Source: CAD feature listing. Evaluate the final solid. Frame: model axes, mm. Give positions to 0.01 mm unless a question says otherwise; leave off trailing zeros. Write each loop counter-clockwise with the first axis right and the second up, starting at its lowest first coordinate (ties: lowest second). Pieces come first, ordered by that corner, then holes. Notation, with made-up numbers: M 20,-6 L 44,-6 A8 ccw 44,-1 Z; hole C 74.5,67.25 d1. An arc over 180 degrees is marked long. Use CSV: the item, a comma, the result in double quotes. Start each with the question number.
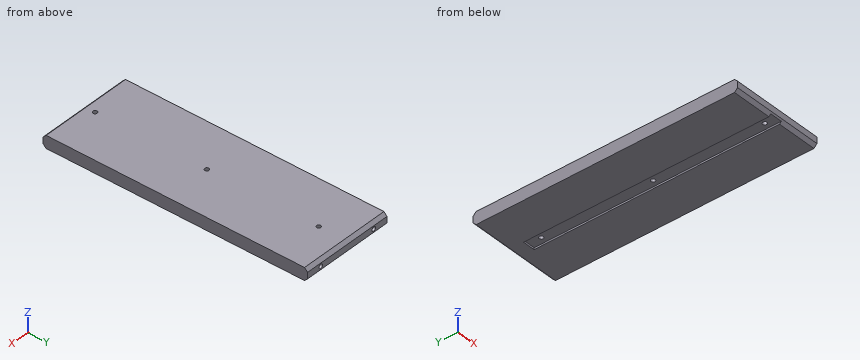
from build123d import *

# Parameters (mm, degrees)
SKETCH1_W             = 150
SKETCH1_H             = 426
BOSS_EXTRUDE1_DEPTH   = 20
SKETCH2_W             = 20
SKETCH2_H             = 400
CUT_EXTRUDE1_DEPTH    = 3
M8_TAPPED_HOLE2_D     = 6.8
M8_TAPPED_HOLE2_DEPTH = 19.75
M8_TAPPED_HOLE2_TIP   = 2.042926105
M8_TAPPED_HOLE1_D     = 6.8
M8_TAPPED_HOLE1_DEPTH = 20
M8_TAPPED_HOLE1_TIP   = 2.042926105
CHAMFER1_SIZE         = 5
CHAMFER2_SIZE         = 5


with BuildPart() as part:
    # Sketch1 → Boss-Extrude1 (new body)
    with BuildSketch(Plane.XY):
        with Locations((75, 213)):
            Rectangle(SKETCH1_W, SKETCH1_H)
    extrude(amount=BOSS_EXTRUDE1_DEPTH)

    # Sketch2 → Cut-Extrude1 (cut)
    with BuildSketch(Plane(origin=(0, 0, 0), x_dir=(-1, 0, 0), z_dir=(0, 0, -1))):
        with Locations((-75, 200)):
            Rectangle(SKETCH2_W, SKETCH2_H)
    extrude(amount=-CUT_EXTRUDE1_DEPTH, mode=Mode.SUBTRACT)

    # M8 Tapped Hole2
    with Locations(Plane(origin=(0, 0, 3), x_dir=(-1, 0, 0), z_dir=(0, 0, -1))):
        with Locations((-75, 20), (-75, 200), (-75, 380)):
            Hole(M8_TAPPED_HOLE2_D / 2, depth=M8_TAPPED_HOLE2_DEPTH)
            with Locations((0, 0, -(M8_TAPPED_HOLE2_DEPTH + M8_TAPPED_HOLE2_TIP / 2))):  # 118° drill point
                Cone(0, M8_TAPPED_HOLE2_D / 2, M8_TAPPED_HOLE2_TIP, mode=Mode.SUBTRACT)

    # M8 Tapped Hole1
    with Locations(Plane(origin=(0, 426, 0), x_dir=(1, 0, 0), z_dir=(0, 1, 0))):
        with Locations((25, -10), (125, -10)):
            Hole(M8_TAPPED_HOLE1_D / 2, depth=M8_TAPPED_HOLE1_DEPTH)
            with Locations((0, 0, -(M8_TAPPED_HOLE1_DEPTH + M8_TAPPED_HOLE1_TIP / 2))):  # 118° drill point
                Cone(0, M8_TAPPED_HOLE1_D / 2, M8_TAPPED_HOLE1_TIP, mode=Mode.SUBTRACT)

    # Chamfer1
    chamfer1_edges = [part.edges().sort_by_distance(p)[0] for p in [
        (75, 0, 20),
        (32.5, 0, 0),
    ]]
    chamfer(chamfer1_edges, length=CHAMFER1_SIZE)

    # Chamfer2
    chamfer2_edges = [part.edges().sort_by_distance(p)[0] for p in [
        (75, 426, 20),
        (75, 426, 0),
    ]]
    chamfer(chamfer2_edges, length=CHAMFER2_SIZE)


solid = part.part
Item 1: Contact query for flat-ended pins moving along their axis: pin 1 Ø3 at (x, z) = (106.5, 17.5) entering from -Y; pin 2 Ø1.5 at (x, z) = (77.5, 1.5) entering from -Y. Output: stop coordinate, or through.
Item 2: Material intervals for probe 1 along Y at (x, z) = (75, 12.75); probe 2 along X at (y, z) = (422.25, 10); probe 3 along X at (y, z) = (166.5, 1.75), sorted ascending.
Item 3: Section A-A (y = 329.5). Return the cut outline in (x, z), plus the area to 3 significant figures.
Output values:
1,pin 1,"stops at y = 1"
1,pin 2,"stops at y = 400"
2,probe 1,"y = 0 to 16.6, 23.4 to 196.6, 203.4 to 376.6, 383.4 to 426"
2,probe 2,"x = 0 to 21.6, 28.4 to 121.6, 128.4 to 150"
2,probe 3,"x = 0 to 65, 85 to 150"
3,outline,"M 0,0 L 65,0 L 65,3 L 85,3 L 85,0 L 150,0 L 150,20 L 0,20 Z"
3,area,"2,940 mm2"
